from build123d import *

# Parameters (mm, degrees)
SKETCH_1_W          = 168
SKETCH_1_H          = 68.565713714
EXTRUDE_1_DEPTH     = 10
SKETCH_2_R          = 4
SKETCH_2_R_2        = 5
CUT_EXTRUDE_1_DEPTH = 10
FILLET_1_R          = 20


with BuildPart() as part:
    # 草图1 → 凸台-拉伸1 (new body)
    with BuildSketch(Plane.XY):
        with Locations((0, -80)):
            Rectangle(SKETCH_1_W, SKETCH_1_H)
    extrude(amount=-EXTRUDE_1_DEPTH)

    # 草图2 → 切除-拉伸1 (cut)
    with BuildSketch(Plane.XY):
        with Locations((-70, -60)):
            Circle(SKETCH_2_R)
        with Locations((-70, -100)):
            Circle(SKETCH_2_R_2)
        with Locations((70, -60)):
            Circle(SKETCH_2_R_2)
        with Locations((70, -100)):
            Circle(SKETCH_2_R_2)
    extrude(amount=-CUT_EXTRUDE_1_DEPTH, mode=Mode.SUBTRACT)

    # 圆角1
    fillet_1_edges = [part.edges().sort_by_distance(p)[0] for p in [
        (-84, -45.717143143, -5),
        (84, -45.717143143, -5),
        (84, -114.282856857, -5),
        (-84, -114.282856857, -5),
    ]]
    fillet(fillet_1_edges, radius=FILLET_1_R)


solid = part.part
Could you check a few things on this model? Use its own coordinates, in mm. Coordinates: 2 decimals unless noted, no trailing zeros. Order: outer loops, then holes, each group sorted by start corner. A loop starts at its lowest first (then second) coordinate and runs counter-clockwise, first axis right, second up. Notation, with made-up numbers: (-33.5, 13) - (23.5, 13) arc R23 cw to (23.5, 31) - close; hole circle Ø5 at (1, -20.75). An arc over 180 degrees is marked (long way). Answer in a Markdown table with one row per item. Add a question column.
(1) If we section it at B-B, the plane z = -6.5: Please give me the cut outline in (x, y), then the cut area to 3 significant figures.
(2) If we section it at C-C, the plane y = -60: Please give me the cut outline in (x, z).
(3) Will these pins go through, and if not, where does the flat tip stop? pin 1 (1.5 mm diameter, centred on y = -95.5, z = -6, fed in from +X); pin 2 (6 mm diameter, centred on y = -105.5, z = -7, fed in from -X); pin 3 (13 mm diameter, centred on x = -70, y = -100, fed in from +Z); pin 4 (4 mm diameter, centred on y = -59.5, z = -6, fed in from -X).
(4) If we section it at A-A, the plane x = -72: Please give me the cut outline in (y, z), then the cut area to 3 significant figures.
(5) If we mould it in two halves opening along Y, with no side actions, what happens to faces 1 (the face through (74.619, -101.915, -4.93)), 2 (the face through (84, -80, -5)), 3 (the face through (-65.381, -101.915, -4.93)), 4 (the face through (77.986, -51.42, -5.07))? For each: released by +Y, released by -Y, zero draft, split by the parting line, or undercut.
(6) I need wall thicknesses on L1, parallel to Y at x = 70, z = -4.75; L2, parallel to X at y = -96, z = -7.75; L3, parallel to Y at x = -70, z = -7.25. Which ranges of each line are inside material? Lowest first, please.
Results are:
| question | item | result |
|---|---|---|
| 1 | outline | (-84, -94.28) arc R20 ccw to (-64, -114.28) - (64, -114.28) arc R20 ccw to (84, -94.28) - (84, -65.72) arc R20 ccw to (64, -45.72) - (-64, -45.72) arc R20 ccw to (-84, -65.72) - close; hole circle Ø10 at (-70, -100); hole circle Ø8 at (-70, -60); hole circle Ø10 at (70, -100); hole circle Ø10 at (70, -60) |
| 1 | area | 10,900 mm2 |
| 2 | outline | (-83.17, -10) - (-74, -10) - (-74, 0) - (-83.17, 0) - close; (-66, -10) - (65, -10) - (65, 0) - (-66, 0) - close; (75, -10) - (83.17, -10) - (83.17, 0) - (75, 0) - close |
| 3 | pin 1 | stops at x = 83.99 |
| 3 | pin 2 | stops at x = -82.23 |
| 3 | pin 3 | stops at z = 0 |
| 3 | pin 4 | stops at x = -83.55 |
| 4 | outline | (-112.61, -10) - (-104.58, -10) - (-104.58, 0) - (-112.61, 0) - close; (-95.42, -10) - (-63.46, -10) - (-63.46, 0) - (-95.42, 0) - close; (-56.54, -10) - (-47.39, -10) - (-47.39, 0) - (-56.54, 0) - close |
| 4 | area | 491 mm2 |
| 5 | face 1 | undercut |
| 5 | face 2 | zero draft |
| 5 | face 3 | undercut |
| 5 | face 4 | released by +Y |
| 6 | L1 | y = -113.36 to -105, -95 to -65, -55 to -46.64 |
| 6 | L2 | x = -83.93 to -73, -67 to 67, 73 to 83.93 |
| 6 | L3 | y = -113.36 to -105, -95 to -64, -56 to -46.64 |
